Here's how the part is built. I have some questions about the finished solid (model axes, mm). A direction names the side the tool comes from. Round coordinates to 2 decimals unless told otherwise and drop trailing zeros. Write each loop counter-clockwise with the first axis right and the second up, starting at its lowest first coordinate (ties: lowest second). Pieces come first, ordered by that corner, then holes. Notation, with made-up numbers: M 62.25,53.25 L 111.25,53.25 A34 cw 111.25,86.25 Z; hole C -7,28 d2. An arc over 180 degrees is marked long. Use a Markdown table: item, result. Add a question column.
```python
from build123d import *

# Parameters (mm, degrees)
SKETCH1_R               = 109.5
SKETCH1_R_2             = 101.5
BOSS_EXTRUDE1_DEPTH     = 150
CUT_EXTRUDE1_REACH      = 217.593
CUT_EXTRUDE1_END_RADIUS = 109.5


with BuildPart() as part:
    # Sketch1 → Boss-Extrude1 (new body)
    with BuildSketch(Plane(origin=(0, 0, 0), x_dir=(1, 0, 0), z_dir=(0, 1, 0))):
        with Locations(Location((0, 0, 0), (0, 0, 270))):
            Circle(SKETCH1_R)
        with Locations(Location((0, 0, 0), (0, 0, 270))):
            Circle(SKETCH1_R_2, mode=Mode.SUBTRACT)
    extrude(amount=BOSS_EXTRUDE1_DEPTH)

    # Cut-Extrude1: up to this cylinder (the profile starts inside it)
    cut_extrude1_end = Plane(origin=(0, 35, 0), z_dir=(0, -1, 0)) * Cylinder(CUT_EXTRUDE1_END_RADIUS, 655.186, mode=Mode.PRIVATE)
    # Sketch2 → Cut-Extrude1 (cut, up to the surface)
    with BuildSketch(Plane.XY, mode=Mode.PRIVATE) as cut_extrude1_sk1:
        with BuildLine():
            Line((-50, 0), (-50, 70))
            ThreePointArc((-50, 70), (0, 120), (50, 70))
            Line((50, 70), (50, 0))
            ThreePointArc((50, 0), (0, -50), (-50, 0))
        make_face()
    cut_extrude1_tool1 = extrude(cut_extrude1_sk1.sketch, amount=CUT_EXTRUDE1_REACH, mode=Mode.PRIVATE) & cut_extrude1_end
    add(cut_extrude1_tool1.solids().sort_by_distance((0, 35, 0))[0], mode=Mode.SUBTRACT)


solid = part.part
```
Item 1: For pin 1 Ø2 at (y, z) = (49, -83) entering from +X; pin 2 Ø4 at (y, z) = (28, 41.5) entering from -X; pin 3 Ø7.5 at (y, z) = (34.5, 93) entering from -X, each with a flat end and sliding along its axis, tell me the tip position at first contact or that it passes through.
Item 2: Imagine slicing it at D-D on y = 20.5. List the corners of the cut face in (x, z) for me, plus the area to 3 significant figures.
Item 3: Imagine slicing it at B-B on z = 0. List the corners of the cut face in (x, y) for me.
Item 4: On a 3-axis mill with a long thin cutter (end or side, diameter ignored), from which of +Z, -Z, +X, -X, +Y, -Y can I reach the whole of each face in a straight line? I mean faces 4 (the face through (50, 35, 93)), 5 (the face through (49, 0, -91)). Say none if no direction works.
Item 5: Imagine slicing it at C-C on y = 141. List the corners of the cut face in (x, z) for me.
Item 6: I need wall thicknesses on probe 1 along X at (y, z) = (95, 0); probe 2 along Z at (x, y) = (-66.5, 117.5); probe 3 along X at (y, z) = (96.5, -34). Which ranges of each line are inside material? Lowest first, please. Write a range as from..to.
Item 7: If we mould it in two halves opening along Z, with no side actions, what happens to faces 1 (the face through (-50, 35, 93)), 2 (the face through (4.5, 74, -101.4)), 3 (the face through (4.815, 73.95, -109.394))? For each: +Z half, -Z half, draft (parallel to the pull), parting line (faces both ways), or undercut.
Item 8: Imagine slicing it at A-A on x = 0. List the corners of the cut face in (y, z) for me, plus the area to 3 significant figures.
The answers:
| question | item | result |
|---|---|---|
| 1 | pin 1 | x = 72.57 |
| 1 | pin 2 | x = -102.13 |
| 1 | pin 3 | x = -63.44 |
| 2 | outline | M -50,88.33 L -50,97.42 A109.5 ccw long 50,97.42 L 50,88.33 A101.5 cw long Z |
| 2 | area | 4,470 mm² |
| 3 | outline | M -109.5,0 L -101.5,0 L -101.5,150 L -109.5,150 Z; M 101.5,0 L 109.5,0 L 109.5,150 L 101.5,150 Z |
| 4 | face 4 | +Z, -Y |
| 4 | face 5 | +Z, -Z, +X, -X, -Y |
| 5 | outline | C 0,0 d219; hole C 0,0 d203 |
| 6 | probe 1 | -109.5..-101.5, 101.5..109.5 |
| 6 | probe 2 | -86.99..-76.68, 76.68..86.99 |
| 6 | probe 3 | -104.09..-95.64, 95.64..104.09 |
| 7 | face 1 | draft |
| 7 | face 2 | undercut |
| 7 | face 3 | parting line |
| 8 | outline | M 0,-109.5 L 150,-109.5 L 150,-101.5 L 0,-101.5 Z; M 120,101.5 L 150,101.5 L 150,109.5 L 120,109.5 Z |
| 8 | area | 1,440 mm² |
